```python
from build123d import *

# Parameters (mm, degrees)
SKETCH1_R           = 1.6
BOSS_EXTRUDE1_DEPTH = 6


with BuildPart() as part:
    # Sketch1 → Boss-Extrude1 (new body)
    with BuildSketch(Plane.XY):
        with BuildLine():
            Line((-45.309203126, -10.68796842), (-43.492395524, -11.905920573))
            ThreePointArc((-43.492395524, -11.905920573), (-42.764262434, -12.595973377), (-42.304336877, -13.487499682))
            ThreePointArc((-42.304336877, -13.487499682), (0.05, -44.45), (42.404336877, -13.487499682))
            ThreePointArc((42.404336877, -13.487499682), (42.864262434, -12.595973377), (43.592395524, -11.905920573))
            Line((43.592395524, -11.905920573), (45.409203126, -10.68796842))
            ThreePointArc((45.409203126, -10.68796842), (46.243586183, -9.847021456), (46.68737785, -8.748642725))
            ThreePointArc((46.68737785, -8.748642725), (47.5, 0), (46.68737785, 8.748642725))
            ThreePointArc((46.68737785, 8.748642725), (46.243586183, 9.847021456), (45.409203126, 10.68796842))
            Line((45.409203126, 10.68796842), (43.592395524, 11.905920573))
            ThreePointArc((43.592395524, 11.905920573), (42.864262434, 12.595973377), (42.404336877, 13.487499682))
            ThreePointArc((42.404336877, 13.487499682), (0.05, 44.45), (-42.304336877, 13.487499682))
            ThreePointArc((-42.304336877, 13.487499682), (-42.764262434, 12.595973377), (-43.492395524, 11.905920573))
            Line((-43.492395524, 11.905920573), (-45.309203126, 10.68796842))
            ThreePointArc((-45.309203126, 10.68796842), (-46.143586183, 9.847021456), (-46.58737785, 8.748642725))
            ThreePointArc((-46.58737785, 8.748642725), (-47.4, 0), (-46.58737785, -8.748642725))
            ThreePointArc((-46.58737785, -8.748642725), (-46.143586183, -9.847021456), (-45.309203126, -10.68796842))
        make_face()
        with Locations((-35.695198541, 20.6375)):
            Circle(SKETCH1_R, mode=Mode.SUBTRACT)
        with Locations((-35.695198541, -20.6375)):
            Circle(SKETCH1_R, mode=Mode.SUBTRACT)
        with Locations((35.795198541, -20.6375)):
            Circle(SKETCH1_R, mode=Mode.SUBTRACT)
        with Locations((35.795198541, 20.6375)):
            Circle(SKETCH1_R, mode=Mode.SUBTRACT)
        with Locations((0.05, -41.275)):
            Circle(SKETCH1_R, mode=Mode.SUBTRACT)
        with Locations((0.05, 41.275)):
            Circle(SKETCH1_R, mode=Mode.SUBTRACT)
    extrude(amount=BOSS_EXTRUDE1_DEPTH)


solid = part.part
```
The model under review builds one solid part; all positions refer to its coordinate system, in mm. Round coordinates to 2 decimals unless told otherwise and drop trailing zeros. Order: outer loops, then holes, each group sorted by start corner. A loop starts at its lowest first (then second) coordinate and runs counter-clockwise, first axis right, second up. Notation, with made-up numbers: M 7,75 L 60,75 A7 cw 60,82 Z; hole C -37,42 d7. An arc over 180 degrees is marked long. Use a Markdown table: item, result.
1) Insertion check: pin 1 (3 mm diameter, centred on x = -35.7, y = -20.64, fed in from -Z); pin 2 (2 mm diameter, centred on x = 8, z = 4, fed in from -Y); pin 3 (3 mm diameter, centred on y = 5.5, z = 4.5, fed in from -X); pin 4 (3 mm diameter, centred on y = -31.5, z = 1, fed in from +X). Each pin has a flat end and moves straight along its axis. Give the tip position at first contact, or say it passes through.
Report:
| item | result |
|---|---|
| pin 1 | through |
| pin 2 | y = -43.9 |
| pin 3 | x = -47.23 |
| pin 4 | x = 32.85 |
2) Draft analysis for pull direction X (two halves, no side actions). For faces 1 (the face through (-0.736, -44.443, 2.958)), 2 (the face through (47.5, -0.1, 3)), 3 (the face through (0.91, 42.624, 2.958)), 4 (the face through (-36.96, 19.66, 2.96)), state which applies: released by +X, released by -X, zero draft, split by the parting line, or undercut.
Report:
| item | result |
|---|---|
| face 1 | split by the parting line |
| face 2 | released by +X |
| face 3 | undercut |
| face 4 | undercut |
3) Consider section A-A (x = 0.05). Write out the cut boundary in (y, z) (3 decimals).
Report:
| item | result |
|---|---|
| outline | M -44.45,0 L -42.875,0 L -42.875,6 L -44.45,6 Z; M -39.675,0 L 39.675,0 L 39.675,6 L -39.675,6 Z; M 42.875,0 L 44.45,0 L 44.45,6 L 42.875,6 Z |
4) Consider section B-B (z = 2.95). Give the number of separate pieces and of enclosed holes in the cut face, then the cut area to 3 significant figures.
Report:
| item | result |
|---|---|
| separate pieces | 1 |
| enclosed holes | 6 |
| area | 6,290 mm^2 |
5) Wall thickness on line 1 along Y through (x, z) = (0.05, 3.65) (3 decimals); line 2 along X through (y, z) = (-21, 3.95); line 3 along X through (y, z) = (-22, 5.5): over which ranges is each line inside the solid? List them lowest first. Write a range as [from, to].
Report:
| item | result |
|---|---|
| line 1 | [-44.45, -42.875], [-39.675, 39.675], [42.875, 44.45] |
| line 2 | [-39.13, -37.25], [-34.14, 34.24], [37.35, 39.23] |
| line 3 | [-38.57, -36.53], [-34.86, 34.96], [36.63, 38.67] |
6) Consider section C-C (y = 17). Write out the cut boundary in (x, z), then the cut area to 3 significant figures.
Report:
| item | result |
|---|---|
| outline | M -41.02,0 L 41.12,0 L 41.12,6 L -41.02,6 Z |
| area | 493 mm^2 |
7) Consider section D-D (x = -23). Write out the cut boundary in (y, z).
Report:
| item | result |
|---|---|
| outline | M -38.01,0 L 38.01,0 L 38.01,6 L -38.01,6 Z |
